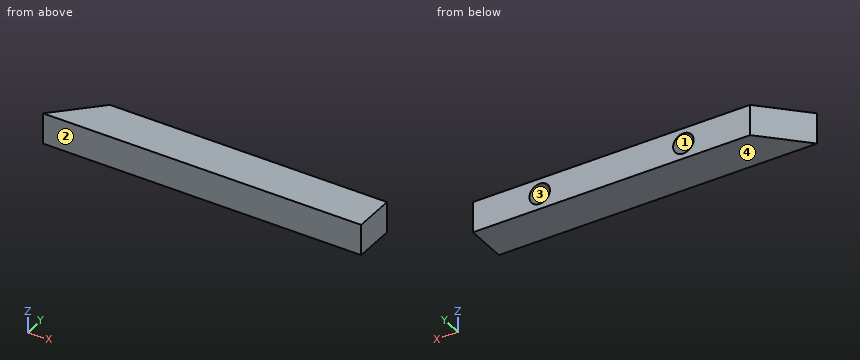
from build123d import *

# Parameters (mm, degrees)
SKETCH_1_W          = 270
SKETCH_1_H          = 30
EXTRUDE_1_DEPTH     = 40
SKETCH_2_R          = 10
CUT_EXTRUDE_2_DEPTH = 30
SKETCH_3_W          = 30
SKETCH_3_H          = 40
EXTRUDE_2_DEPTH     = 40
CUT_EXTRUDE_3_DEPTH = 183.002747232


with BuildPart() as part:
    # 草图1 → 凸台-拉伸1 (new body)
    with BuildSketch(Plane(origin=(0, 0, 0), x_dir=(1, 0, 0), z_dir=(0, 1, 0))):
        Rectangle(SKETCH_1_W, SKETCH_1_H)
    extrude(amount=EXTRUDE_1_DEPTH)

    # 草图2 → 切除-拉伸2 (cut)
    with BuildSketch(Plane(origin=(0, 40, 0), x_dir=(1, 0, 0), z_dir=(0, 1, 0))):
        with Locations(Location((70, 0, 0), (0, 0, 270))):
            Circle(SKETCH_2_R)
        with Locations(Location((-70, 0, 0), (0, 0, 90))):
            Circle(SKETCH_2_R)
    extrude(amount=-CUT_EXTRUDE_2_DEPTH, mode=Mode.SUBTRACT)

    # 草图3 → 凸台-拉伸2 (add)
    with BuildSketch(Plane.ZY.offset(135)):
        with Locations((0, 20)):
            Rectangle(SKETCH_3_W, SKETCH_3_H)
    extrude(amount=EXTRUDE_2_DEPTH)

    # 草图4 → 切除-拉伸3 (cut, through all)
    with BuildSketch(Plane.XY.offset(15)):
        Polygon((-175, 0), (-135, 40), (-175, 40), align=None)
    extrude(amount=-CUT_EXTRUDE_3_DEPTH, mode=Mode.SUBTRACT)


solid = part.part
The listing builds one solid part. Answer for the finished solid, in the listing's coordinates (mm). Face numbers are marked on the shaded views. Give positions to 0.01 mm unless a question says otherwise; leave off trailing zeros. Write each loop counter-clockwise with the first axis right and the second up, starting at its lowest first coordinate (ties: lowest second). Pieces come first, ordered by that corner, then holes. Notation, with made-up numbers: (-8, -18.75) - (35, -18.75) arc R20 cw to (35, 13.25) - close; hole circle Ø4 at (54.25, -24). An arc over 180 degrees is marked (long way). Use a Markdown table: item, result.
1. Section C-C on x = -70 is taken. Write down the section's boundary in (y, z), plus the area to 3 significant figures.
Values follow:
| item | result |
|---|---|
| outline | (0, -15) - (40, -15) - (40, -10) - (10, -10) - (10, 10) - (40, 10) - (40, 15) - (0, 15) - close |
| area | 600 mm² |
2. Each of these flat-tipped pins is pushed along its axis until it touches: P1, Ø10, axis at y = 33, z = 3, coming from the -X side; P2, Ø6, axis at x = 70.5, z = 2, coming from the +Y side. Where does it stop, or does it pass through?
Values follow:
| item | result |
|---|---|
| P1 | stops at x = -147 |
| P2 | stops at y = 10 |
3. Section A-A on y = 33.5 is taken. Write down the section's boundary in (x, z), plus the area to 3 significant figures.
Values follow:
| item | result |
|---|---|
| outline | (-141.5, -15) - (135, -15) - (135, 15) - (-141.5, 15) - close; hole circle Ø20 at (-70, 0); hole circle Ø20 at (70, 0) |
| area | 7,670 mm² |
4. For a pull along Z with two mould halves and no side action, classify the marked faces 1, 2, 3 and 4 as released by +Z, released by -Z, zero draft, split by the parting line, or undercut.
Values follow:
| item | result |
|---|---|
| face 1 | undercut |
| face 2 | zero draft |
| face 3 | undercut |
| face 4 | released by -Z |
5. Section D-D on y = 5 is taken. Write down the section's boundary in (x, z), plus the area to 3 significant figures.
Values follow:
| item | result |
|---|---|
| outline | (-170, -15) - (135, -15) - (135, 15) - (-170, 15) - close |
| area | 9,150 mm² |
6. Section B-B on z = 0 is taken. Write down the section's boundary in (x, y).
Values follow:
| item | result |
|---|---|
| outline | (-175, 0) - (135, 0) - (135, 40) - (80, 40) - (80, 10) - (60, 10) - (60, 40) - (-60, 40) - (-60, 10) - (-80, 10) - (-80, 40) - (-135, 40) - close |
7. Find the intervals of material crossed by probe 1 along X at (y, z) = (25, 6.5); probe 2 along X at (y, z) = (29, -9); probe 3 along Z at (x, y) = (77, 20), in increasing order. Write a range as from..to.
Values follow:
| item | result |
|---|---|
| probe 1 | x = -150..-77.6, -62.4..62.4, 77.6..135 |
| probe 2 | x = -146..-74.36, -65.64..65.64, 74.36..135 |
| probe 3 | z = -15..-7.14, 7.14..15 |
